The model under review builds one solid part; all positions refer to its coordinate system, in mm. A direction names the side the tool comes from. Coordinates: 2 decimals unless noted, no trailing zeros. Write each loop counter-clockwise with the first axis right and the second up, starting at its lowest first coordinate (ties: lowest second). Pieces come first, ordered by that corner, then holes. Notation, with made-up numbers: (89.25, 43.5) - (120.25, 43.5) arc R26 cw to (120.25, 77.5) - close; hole circle Ø1 at (20.25, -18). An arc over 180 degrees is marked (long way). Put each result on its own line as item: value.
from build123d import *

# Parameters (mm, degrees)
BODY_PROFILE_35_R             = 17.5
BODY_35_DEPTH                 = 15
FLANGE_PROFILE_45_R           = 22.5
FLANGE_45_DEPTH               = 5
BODY_END_CHAMFER_0_8X60_SIZE  = 0.8
BODY_END_CHAMFER_0_8X60_SIZE2 = 1.385640646
BORE_PROFILE_25_R             = 12.5
BORE_25_DEPTH                 = 38.583240946
FLANGE_BORE_FILLET_R2_R       = 2
FLANGE_EDGE_CHAMFER_1X45_SIZE = 1
BODY_BORE_FILLET_R1_R         = 1


with BuildPart() as part:
    # Body Profile Ø35 → Body Ø35 (new body)
    with BuildSketch(Plane.XY):
        Circle(BODY_PROFILE_35_R)
    extrude(amount=BODY_35_DEPTH)

    # Flange Profile Ø45 → Flange Ø45 (add)
    with BuildSketch(Plane.XY.offset(15)):
        Circle(FLANGE_PROFILE_45_R)
    extrude(amount=FLANGE_45_DEPTH)

    # Body End Chamfer 0.8x60°
    body_end_chamfer_0_8x60_edges = [part.edges().sort_by_distance(p)[0] for p in [
        (-17.5, 0, 0),
    ]]
    body_end_chamfer_0_8x60_side = [part.faces().sort_by_distance(p)[0] for p in [
        (0, 0, 0),
    ]]
    chamfer(body_end_chamfer_0_8x60_edges, length=BODY_END_CHAMFER_0_8X60_SIZE, length2=BODY_END_CHAMFER_0_8X60_SIZE2, reference=body_end_chamfer_0_8x60_side[0])

    # Bore Profile Ø25 → Bore Ø25 (cut, through all)
    with BuildSketch(Plane.XY.offset(20)):
        Circle(BORE_PROFILE_25_R)
    extrude(amount=-BORE_25_DEPTH, mode=Mode.SUBTRACT)

    # Flange Bore Fillet R2
    flange_bore_fillet_r2_edges = [part.edges().sort_by_distance(p)[0] for p in [
        (-12.5, 0, 20),
    ]]
    fillet(flange_bore_fillet_r2_edges, radius=FLANGE_BORE_FILLET_R2_R)

    # Flange Edge Chamfer 1x45°
    flange_edge_chamfer_1x45_edges = [part.edges().sort_by_distance(p)[0] for p in [
        (-22.5, 0, 15),
        (-22.5, 0, 20),
    ]]
    chamfer(flange_edge_chamfer_1x45_edges, length=FLANGE_EDGE_CHAMFER_1X45_SIZE)

    # Body Bore Fillet R1
    body_bore_fillet_r1_edges = [part.edges().sort_by_distance(p)[0] for p in [
        (-12.5, 0, 0),
    ]]
    fillet(body_bore_fillet_r1_edges, radius=BODY_BORE_FILLET_R1_R)


solid = part.part
1. Consider section C-C on z = 13.5. State the section outline as (x, y) points, plus the area to 3 significant figures.
Determined:
outline: circle Ø35 at (0, 0); hole circle Ø25 at (0, 0)
area: 471 mm^2
2. For pin 1 Ø12 at (x, z) = (-0.5, 10.5) entering from -Y; pin 2 Ø12 at (x, z) = (-0.5, 18) entering from +Y; pin 3 Ø4 at (x, z) = (-1.5, 2.5) entering from -Y; pin 4 Ø1 at (x, y) = (15.5, -17.5) entering from +Z, all flat-tipped, find the tip position at first contact; note any pin that passes through.
Determined:
pin 1: stops at y = -22.5
pin 2: stops at y = 22.5
pin 3: stops at y = -17.5
pin 4: passes through
3. To check wall thickness, follow probe 1 along Y at (x, z) = (0, 9.5); probe 2 along Y at (x, z) = (4, 7.25); probe 3 along X at (y, z) = (-11, 1.5). State the ranges of each line that lie inside material, in increasing order.
Determined:
probe 1: y = -17.5 to -12.5, 12.5 to 17.5
probe 2: y = -17.04 to -11.84, 11.84 to 17.04
probe 3: x = -13.61 to -5.94, 5.94 to 13.61
4. The part is to be moulded in two halves that separate along Y. For faces 1 (the flat face through (14, 0, 0)), 2 (the cylindrical face through (11.923, 3.755, 9.619)), 3 (the cylindrical face through (10.382, -19.961, 17.479)), say which applies: +Y half, -Y half, draft (parallel to the pull), parting line (faces both ways), or undercut.
Determined:
face 1: draft
face 2: undercut
face 3: parting line
5. Machinability: for faces 4 (the flat face through (14, -4.5, 20)), 5 (the cylindrical face through (-13.887, -10.648, 8.098)), which of the approach directions +Z, -Z, +X, -X, +Y, -Y give a long, thin tool a straight path to every point of the face, cutting with its end or side? Answer none if there is none.
Determined:
face 4: +Z, +X, -X, +Y, -Y
face 5: -Z
6. Consider section A-A on x = 0. State the section outline as (y, z) points, plus the area to 3 significant figures.
Determined:
outline: (-22.5, 16) - (-21.5, 15) - (-17.5, 15) - (-17.5, 1.39) - (-16.7, 0) - (-13.5, 0) arc R1 ccw to (-12.5, 1) - (-12.5, 18) arc R2 ccw to (-14.5, 20) - (-21.5, 20) - (-22.5, 19) - close; (12.5, 1) arc R1 ccw to (13.5, 0) - (16.7, 0) - (17.5, 1.39) - (17.5, 15) - (21.5, 15) - (22.5, 16) - (22.5, 19) - (21.5, 20) - (14.5, 20) arc R2 ccw to (12.5, 18) - close
area: 245 mm^2
